Drawing for the job (mm, zero at the part's lowest x, y, z). A direction names the side the tool comes from. Coordinates: 2 decimals unless noted, no trailing zeros. Order: outer loops, then holes, each group sorted by start corner. A loop starts at its lowest first (then second) coordinate and runs counter-clockwise, first axis right, second up. Notation, with made-up numbers: (18, 4.25) - (32, 4.25) arc R7 ccw to (32, 13.25) - close; hole circle Ø3 at (-10, -14.5). An arc over 180 degrees is marked (long way). Answer as CSV lines item,"result". Start each with the question number.
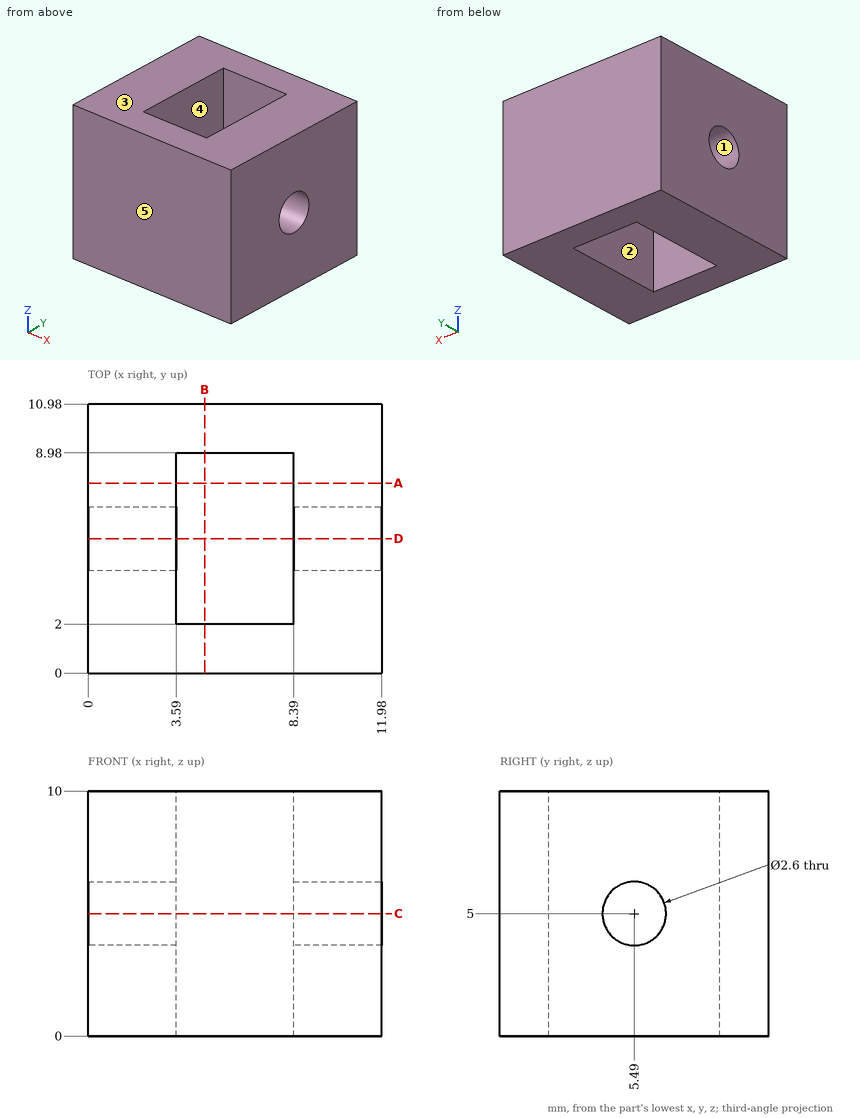
(1) Band-saw the part on C-C on z = 5. List the corners of the cut face in (x, y), plus the area to 3 significant figures.
(2) Band-saw the part on B-B on x = 4.75. List the corners of the cut face in (y, z), plus the area to 3 significant figures.
(3) Band-saw the part on A-A on y = 7.75. List the corners of the cut face in (x, z), plus the area to 3 significant figures.
(4) Which spindle directions (+Z, -Z, +X, -X, +Y, -Y) get a long thin tool onto all of the face, cutting with end or side? Do the marked faces 1 and 2. Say none if no direction does.
(5) Pull direction Y, two halves, no side cores. Call the marked faces 3, 4 and 5: +Y half, -Y half, draft (parallel to the pull), parting line (faces both ways), or undercut.
(6) Probe L1, parallel to X at y = 4.5, z = 8; L2, parallel to Y at x = 2.25, z = 5; L3, parallel to Y at x = 4.25, z = 9.25. List the from-to ranges inside material, lowest first. Write a range as [from, to].
(7) Band-saw the part on D-D on y = 5.49. List the corners of the cut face in (x, z), plus the area to 3 significant figures.
(8) Drop flat-ended pins along their axis: pin 1 Ø2 at (y, z) = (5.5, 3.5) entering from -X; pin 2 Ø2.5 at (y, z) = (5.49, 5) entering from +X. Give the stop position or say it passes through.
Filled in:
1,outline,"(0, 0) - (11.98, 0) - (11.98, 4.19) - (8.39, 4.19) - (8.39, 2) - (3.59, 2) - (3.59, 4.19) - (0, 4.19) - close; (0, 6.79) - (3.59, 6.79) - (3.59, 8.98) - (8.39, 8.98) - (8.39, 6.79) - (11.98, 6.79) - (11.98, 10.98) - (0, 10.98) - close"
1,area,"79.4 mm^2"
2,outline,"(0, 0) - (2, 0) - (2, 10) - (0, 10) - close; (8.98, 0) - (10.98, 0) - (10.98, 10) - (8.98, 10) - close"
2,area,"40.0 mm^2"
3,outline,"(0, 0) - (3.59, 0) - (3.59, 10) - (0, 10) - close; (8.39, 0) - (11.98, 0) - (11.98, 10) - (8.39, 10) - close"
3,area,"71.8 mm^2"
4,face 1,"+X, -X"
4,face 2,"+Z, -Z"
5,face 3,"draft"
5,face 4,"undercut"
5,face 5,"-Y half"
6,L1,"x = [0, 3.59], [8.39, 11.98]"
6,L2,"y = [0, 4.19], [6.79, 10.98]"
6,L3,"y = [0, 2], [8.98, 10.98]"
7,outline,"(0, 0) - (3.59, 0) - (3.59, 3.7) - (0, 3.7) - close; (0, 6.3) - (3.59, 6.3) - (3.59, 10) - (0, 10) - close; (8.39, 0) - (11.98, 0) - (11.98, 3.7) - (8.39, 3.7) - close; (8.39, 6.3) - (11.98, 6.3) - (11.98, 10) - (8.39, 10) - close"
7,area,"53.1 mm^2"
8,pin 1,"stops at x = 0"
8,pin 2,"passes through"
